from build123d import *

# Parameters (mm, degrees)
SKETCH1_W             = 20
SKETCH1_H             = 8
BOSS_EXTRUDE1_DEPTH   = 39.9
SKETCH2_W             = 9
SKETCH2_H             = 9
CUT_EXTRUDE1_DEPTH    = 42.328077623
CHAMFER1_SIZE         = 0.3
SKETCH3_R             = 0.5930201
CUT_EXTRUDE2_DEPTH    = 3
SKETCH4_R             = 0.6
CUT_EXTRUDE3_DEPTH    = 4.5
M3_TAPPED_HOLE1_D     = 2.5
M3_TAPPED_HOLE1_DEPTH = 5
M3_TAPPED_HOLE1_TIP   = 0.751075774


with BuildPart() as part:
    # Sketch1 → Boss-Extrude1 (new body)
    with BuildSketch(Plane(origin=(0, 0, 0), x_dir=(1, 0, 0), z_dir=(0, 1, 0))):
        Rectangle(SKETCH1_W, SKETCH1_H)
    extrude(amount=BOSS_EXTRUDE1_DEPTH)

    # Sketch2 → Cut-Extrude1 (cut, through all)
    with BuildSketch(Plane(origin=(0, 39.9, 0), x_dir=(1, 0, 0), z_dir=(0, 1, 0))):
        with Locations((0, -4)):
            Rectangle(SKETCH2_W, SKETCH2_H)
    extrude(amount=-CUT_EXTRUDE1_DEPTH, mode=Mode.SUBTRACT)

    # Chamfer1
    chamfer1_edges = [part.edges().sort_by_distance(p)[0] for p in [
        (-10, 19.95, -4),
        (10, 19.95, -4),
    ]]
    chamfer(chamfer1_edges, length=CHAMFER1_SIZE)

    # Sketch3 → Cut-Extrude2 (cut)
    with BuildSketch(Plane(origin=(0, 0, -4), x_dir=(-1, 0, 0), z_dir=(0, 0, -1))):
        with Locations((-7.5, 27.95)):
            Circle(SKETCH3_R)
        with Locations(Location((7.5, 27.95, 0), (0, 0, 180))):
            Circle(SKETCH3_R)
        with Locations((7.5, 11.95)):
            Circle(SKETCH3_R)
        with Locations(Location((-7.5, 11.95, 0), (0, 0, 180))):
            Circle(SKETCH3_R)
    extrude(amount=-CUT_EXTRUDE2_DEPTH, mode=Mode.SUBTRACT)

    # Sketch4 → Cut-Extrude3 (cut)
    with BuildSketch(Plane.XZ):
        with Locations(Location((0, -2.2, 0), (0, 0, 270))):
            Circle(SKETCH4_R)
    extrude(amount=-CUT_EXTRUDE3_DEPTH, mode=Mode.SUBTRACT)

    # M3 Tapped Hole1
    with Locations(Plane(origin=(7.5, 11.95, -4), x_dir=(-1, 0, 0), z_dir=(0, 0, -1))):
        with Locations((0, 0), (15, 0), (15, 16), (0, 16)):
            Hole(M3_TAPPED_HOLE1_D / 2, depth=M3_TAPPED_HOLE1_DEPTH)
            with Locations((0, 0, -(M3_TAPPED_HOLE1_DEPTH + M3_TAPPED_HOLE1_TIP / 2))):  # 118° drill point
                Cone(0, M3_TAPPED_HOLE1_D / 2, M3_TAPPED_HOLE1_TIP, mode=Mode.SUBTRACT)


solid = part.part
Model file for the job. Use its own axes, mm. A direction names the side the tool comes from. Give positions to 0.01 mm unless a question says otherwise; leave off trailing zeros. Order: outer loops, then holes, each group sorted by start corner. A loop starts at its lowest first (then second) coordinate and runs counter-clockwise, first axis right, second up. Notation, with made-up numbers: M 26.5,68.5 L 62.5,68.5 A16 cw 62.5,94.5 Z; hole C 38.5,-10.75 d10. An arc over 180 degrees is marked long. Write item = value, one per line.
Q1. Cut at C-C, the plane z = -1. List the corners of the cut face in (x, y), then the cut area to 3 significant figures.
Derived:
outline = M -10,0 L 10,0 L 10,39.9 L -10,39.9 Z; hole C -7.5,11.95 d2.5; hole C -7.5,27.95 d2.5; hole C 7.5,11.95 d2.5; hole C 7.5,27.95 d2.5
area = 778 mm2
Q2. Flat gauge pin, fed straight in: pin 1 (2.5 mm diameter, centred on x = 0, y = 26, fed in from +Z). Where does the tip first touch, or does it go through?
Derived:
pin_1 = -0.5
Q3. Drill centre lines: line 1 (Y direction, x = 7.5, z = -2.8); line 2 (X direction, y = 11.95, z = -1.1); line 3 (X direction, y = 27.95, z = -0.1). Where is each one in solid material? Low to high. Write a range as [from, to].
Derived:
line_1 = [0, 10.7], [13.2, 26.7], [29.2, 39.9]
line_2 = [-10, -8.75], [-6.25, 6.25], [8.75, 10]
line_3 = [-10, -8.75], [-6.25, -4.5], [4.5, 6.25], [8.75, 10]
Q4. Two-plate mould, pull along Z, no slides. Class faces 4 (the flat face through (0, 0, -1)), 5 (the cylindrical face through (0.18, 2.218, -2.772)), 6 (the flat face through (7, 20, 4)), 7 (the flat face through (0, 4.5, -2)): pulls with the +Z half, pulls with the -Z half, needs draft (parallel to the pull), parting line crosses it, or undercut.
Derived:
face_4 = needs draft
face_5 = undercut
face_6 = pulls with the +Z half
face_7 = undercut
Q5. Tool access for faces 1 (the flat face through (10, 20, 0)), 2 (the flat face through (0, 20, -0.5)), 3 (the cylindrical face through (-7.77, 26.73, -1.46)): list every direction of +Z, -Z, +X, -X, +Y, -Y with a clear straight run to the whole face (end or side of a thin tool).
Derived:
face_1 = +Z, -Z, +X, +Y, -Y
face_2 = +Z, +Y, -Y
face_3 = -Z
Q6. Cut at D-D, the plane y = 37. List the corners of the cut face in (x, z), then the cut area to 3 significant figures.
Derived:
outline = M -10,-3.7 L -9.7,-4 L 9.7,-4 L 10,-3.7 L 10,4 L 4.5,4 L 4.5,-0.5 L -4.5,-0.5 L -4.5,4 L -10,4 Z
area = 119 mm2
Q7. Cut at B-B, the plane z = 3.25. List the corners of the cut face in (x, y), then the cut area to 3 significant figures.
Derived:
outline = M -10,0 L -4.5,0 L -4.5,39.9 L -10,39.9 Z; M 4.5,0 L 10,0 L 10,39.9 L 4.5,39.9 Z
area = 439 mm2
Q8. Cut at A-A, the plane y = 4. List the corners of the cut face in (x, z), then the cut area to 3 significant figures.
Derived:
outline = M -10,-3.7 L -9.7,-4 L 9.7,-4 L 10,-3.7 L 10,4 L 4.5,4 L 4.5,-0.5 L -4.5,-0.5 L -4.5,4 L -10,4 Z; hole C 0,-2.2 d1.2
area = 118 mm2
